from build123d import *

# Parameters (mm, degrees)
BRACKET_BODY_DEPTH      = 45
UPRIGHT_HOLE_A_SKETCH_R = 6.5
UPRIGHT_HOLE_A_13_DEPTH = 17.5
UPRIGHT_START           = -17.5
UPRIGHT_HOLE_B_SKETCH_R = 6.5
UPRIGHT_HOLE_B_13_DEPTH = 17.5
FLANGE_HOLE_A_SKETCH_R  = 6.5
FLANGE_HOLE_A_13_DEPTH  = 14
FLANGE_HOLE_B_SKETCH_R  = 6.5
FLANGE_HOLE_B_13_DEPTH  = 14


with BuildPart() as part:
    # Bracket Profile Sketch → Bracket Body (new body)
    with BuildSketch(Plane.XY):
        Polygon((0, 0), (42.5, 0), (42.5, 18), (77.5, 18), (77.5, 0), (120, 0), (120, 14), (90, 14), (90, 60), (72.5, 60), (72.5, 35), (47.5, 35), (47.5, 60), (30, 60), (30, 14), (0, 14), align=None)
    extrude(amount=BRACKET_BODY_DEPTH)

    # Upright Hole A Sketch → Upright Hole A Ø13 (cut)
    with BuildSketch(Plane.ZY.offset(-30)):
        with Locations((22.5, 46)):
            Circle(UPRIGHT_HOLE_A_SKETCH_R)
    extrude(amount=-UPRIGHT_HOLE_A_13_DEPTH, mode=Mode.SUBTRACT)

    # Upright Hole B Sketch → Upright Hole B Ø13 (cut)
    with BuildSketch(Plane(origin=(90, 0, 0), x_dir=(0, 0, -1), z_dir=(1, 0, 0)).offset(UPRIGHT_START)):
        with Locations(Location((-22.5, 46, 0), (0, 0, 180))):
            Circle(UPRIGHT_HOLE_B_SKETCH_R)
    extrude(amount=UPRIGHT_HOLE_B_13_DEPTH, mode=Mode.SUBTRACT)

    # Flange Hole A Sketch → Flange Hole A Ø13 (cut)
    with BuildSketch(Plane(origin=(0, 14, 0), x_dir=(1, 0, 0), z_dir=(0, 1, 0))):
        with Locations(Location((14.919656615, -20, 0), (0, 0, 270))):
            Circle(FLANGE_HOLE_A_SKETCH_R)
    extrude(amount=-FLANGE_HOLE_A_13_DEPTH, mode=Mode.SUBTRACT)

    # Flange Hole B Sketch → Flange Hole B Ø13 (cut)
    with BuildSketch(Plane(origin=(0, 14, 0), x_dir=(1, 0, 0), z_dir=(0, 1, 0))):
        with Locations(Location((106.287852583, -20, 0), (0, 0, 270))):
            Circle(FLANGE_HOLE_B_SKETCH_R)
    extrude(amount=-FLANGE_HOLE_B_13_DEPTH, mode=Mode.SUBTRACT)


solid = part.part
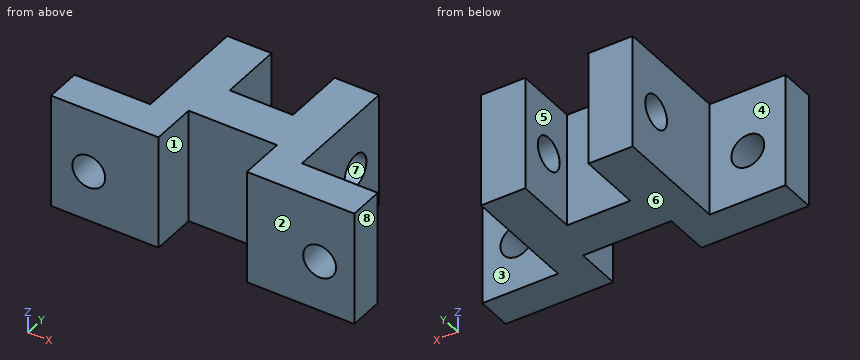
Input: part model. Units: mm. Frame: model coordinates. Face numbers are marked on the shaded views. A direction names the side the tool comes from. Coordinates: 2 decimals unless noted, no trailing zeros. Loops run counter-clockwise (first coordinate to the right, second up) from the corner with the lowest first, then second, coordinate; pieces in that order, holes last. Notation, with made-up numbers: (29.5, 79) - (51.5, 79) arc R8 ccw to (51.5, 88) - close; hole circle Ø5 at (28.5, -24.5). An arc over 180 degrees is marked (long way). Answer in a Markdown table with one row per item. Add a question column.
Item 1: Section query A-A on z = 20. State how many separate pieces and enclosed holes the cut face has, then the cut area to 3 significant figures.
Item 2: Section query D-D on y = 46. Return the cut outline in (x, z), then the cut area to 3 significant figures.
Item 3: Mould query, pull axis Z, two halves, no side actions, for the marked faces 6, 7 and 8. Classes: released by +Z, released by -Z, zero draft, split by the parting line, or undercut.
Item 4: Contact query for flat-ended pins moving along their axis: P1, Ø22.5, axis at y = 41.5, z = 20.5, coming from the -X side; P2, Ø8, axis at x = 100, z = 23.5, coming from the -Y side; P3, Ø3, axis at x = 13.5, z = 13, coming from the +Y side. Output: stop coordinate, or through.
Item 5: Line query: line 1 along X through (y, z) = (7, 20); line 2 along X through (y, z) = (54, 16.5); line 3 along Z through (x, y) = (82, 46). Output: solid intervals per line, ascending. Write a range as [from, to].
Item 6: Access query for the marked faces 1, 2, 3, 4 and 5. Directions: +Z, -Z, +X, -X, +Y, -Y. A direction counts if a zero-diameter tool reaches every point of the face in a straight line with its end or side. Return the directions, or none.
Item 7: Section query B-B on y = 56.5. Return the cut outline in (x, z).
Item 8: Section query C-C on x = 74.5. Return the cut outline in (y, z).
Recorded:
| question | item | result |
|---|---|---|
| 1 | separate pieces | 5 |
| 1 | enclosed holes | 0 |
| 1 | area | 2,400 mm^2 |
| 2 | outline | (30, 0) - (47.5, 0) - (47.5, 16) - (30, 16) - close; (30, 29) - (47.5, 29) - (47.5, 45) - (30, 45) - close; (72.5, 0) - (90, 0) - (90, 16) - (72.5, 16) - close; (72.5, 29) - (90, 29) - (90, 45) - (72.5, 45) - close |
| 2 | area | 1,120 mm^2 |
| 3 | face 6 | released by -Z |
| 3 | face 7 | undercut |
| 3 | face 8 | zero draft |
| 4 | P1 | x = 30 |
| 4 | P2 | y = 0 |
| 4 | P3 | y = 14 |
| 5 | line 1 | [0, 8.42], [21.42, 42.5], [77.5, 99.79], [112.79, 120] |
| 5 | line 2 | [30, 47.5], [72.5, 90] |
| 5 | line 3 | [0, 16], [29, 45] |
| 6 | face 1 | +Z, -Z, -Y |
| 6 | face 2 | +Z, -Z, +X, -X, -Y |
| 6 | face 3 | +Z, -Z, +X, +Y |
| 6 | face 4 | +Z, -Z, -X, +Y |
| 6 | face 5 | +Z, -Z, +Y |
| 7 | outline | (30, 0) - (47.5, 0) - (47.5, 45) - (30, 45) - close; (72.5, 0) - (90, 0) - (90, 45) - (72.5, 45) - close |
| 8 | outline | (18, 0) - (60, 0) - (60, 45) - (18, 45) - close; hole circle Ø13 at (46, 22.5) |
